Here's the drawing with two shaded views (mm, measured from the low corner). I have some questions. Round coordinates to 2 decimals unless told otherwise and drop trailing zeros. Write each loop counter-clockwise with the first axis right and the second up, starting at its lowest first coordinate (ties: lowest second). Pieces come first, ordered by that corner, then holes. Notation, with made-up numbers: (42, 38) - (48, 38) arc R27 cw to (48, 72) - close; hole circle Ø7 at (89, 54). An arc over 180 degrees is marked (long way). Return JSON: item names as keys, results as strings. Group by question number.
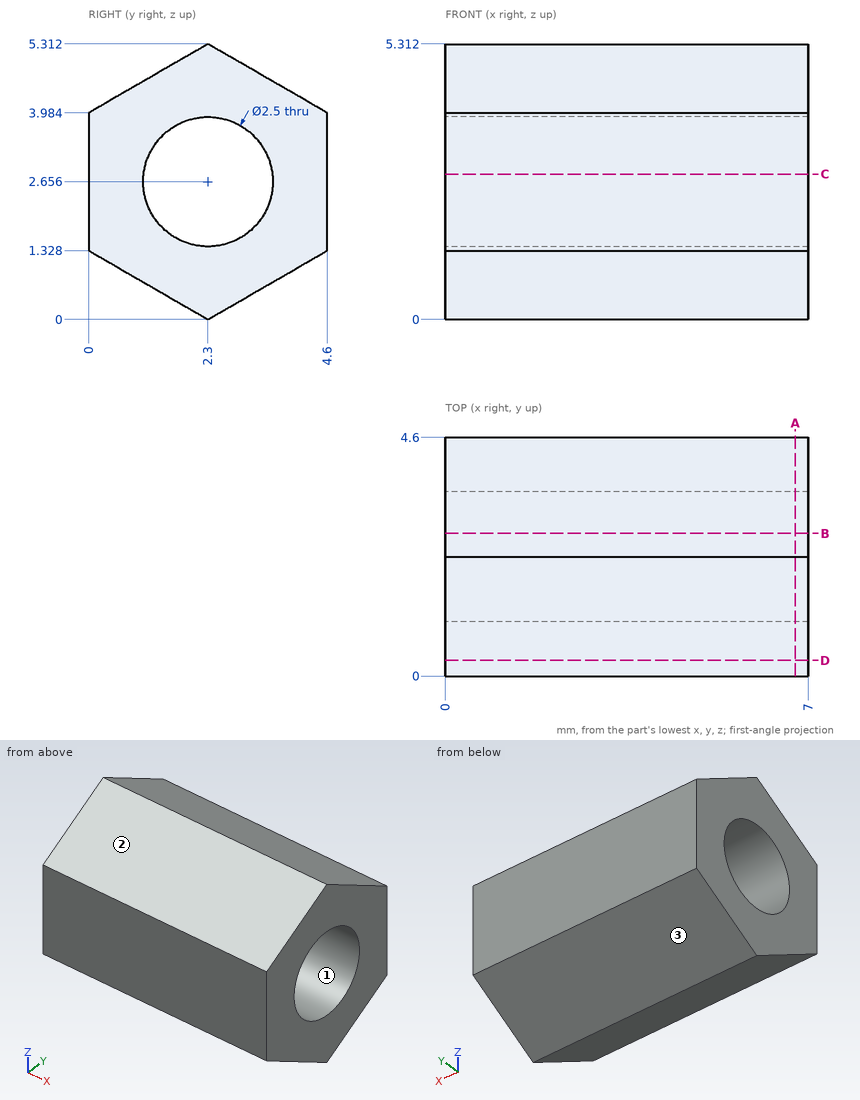
1) I need wall thicknesses on line 1 along Y through (x, z) = (1.75, 3.65) (1 decimal); line 2 along Y through (x, z) = (3.5, 3.4) (1 decimal); line 3 along Z through (x, y) = (2, 2.7). Which ranges of each line are inside material? Lowest first, please.
2) Imagine slicing it at B-B (y = 2.75). Please give me the cut outline in (x, z).
3) Imagine slicing it at A-A (x = 6.75). Please give me the cut outline in (y, z), plus the area to 3 significant figures.
4) If we mould it in two halves opening along Y, with no side actions, what happens to the marked faces 1, 2 and 3? For each: released by +Y, released by -Y, zero draft, split by the parting line, or undercut.
5) Imagine slicing it at C-C (z = 2.8). Please give me the cut outline in (x, y), plus the area to 3 significant figures.
6) Imagine slicing it at D-D (y = 0.3). Please give me the cut outline in (x, z) (1 decimal).
Results found:
{
 "1": {"line 1": "y = 0 to 1.5, 3.1 to 4.6", "line 2": "y = 0 to 1.3, 3.3 to 4.6", "line 3": "z = 0.23 to 1.47, 3.84 to 5.08"},
 "2": {"outline": "(0, 0.26) - (7, 0.26) - (7, 1.49) - (0, 1.49) - close; (0, 3.82) - (7, 3.82) - (7, 5.05) - (0, 5.05) - close"},
 "3": {"outline": "(0, 1.33) - (2.3, 0) - (4.6, 1.33) - (4.6, 3.98) - (2.3, 5.31) - (0, 3.98) - close; hole circle Ø2.5 at (2.3, 2.66)", "area": "13.4 mm²"},
 "4": {"face 1": "undercut", "face 2": "released by -Y", "face 3": "released by +Y"},
 "5": {"outline": "(0, 0) - (7, 0) - (7, 1.06) - (0, 1.06) - close; (0, 3.54) - (7, 3.54) - (7, 4.6) - (0, 4.6) - close", "area": "14.8 mm²"},
 "6": {"outline": "(0, 1.2) - (7, 1.2) - (7, 4.2) - (0, 4.2) - close"}
}
